from build123d import *

# Parameters (mm, degrees)
BASE_BLOCK_DEPTH        = 10
ROUND_SPIGOT_DEPTH      = 9
PROFILE_CUT_A_DEPTH     = 10
TRIANGULAR_POCKET_DEPTH = 10
PROFILE_CUT_B_SKETCH_R  = 0.5
PROFILE_CUT_B_DEPTH     = 5
SPIGOT_CHAMFER_0_5_SIZE = 0.5
SPIGOT_BORE_SKETCH_R    = 1.25
SPIGOT_BORE_DEPTH       = 12
BORE_CHAMFER_1_SIZE     = 1


with BuildPart() as part:
    # Base Block Sketch → Base Block (new body)
    with BuildSketch(Plane.XY):
        Polygon((0, 0), (10, 0), (10, -8), (0, -10), align=None)
    extrude(amount=BASE_BLOCK_DEPTH)

    # Spigot Sketch → Round Spigot (add)
    with BuildSketch(Plane.XY.offset(10)):
        with BuildLine():
            ThreePointArc((5, -0.901174016), (2, -3.901174016), (5, -6.901174016))
            Line((5, -6.901174016), (5, -3.901174016))
            Line((5, -3.901174016), (5, -0.901174016))
        make_face()
        with BuildLine():
            Line((5, -3.901174016), (5, -6.901174016))
            ThreePointArc((5, -6.901174016), (5.282604808, -6.887833442), (5.562696209, -6.847930365))
            Line((5.562696209, -6.847930365), (5, -3.901174016))
        make_face()
        with BuildLine():
            Line((5, -3.901174016), (5.562696209, -6.847930365))
            ThreePointArc((5.562696209, -6.847930365), (7.311718909, -5.813229373), (8, -3.901174016))
            ThreePointArc((8, -3.901174016), (7.121320344, -1.779853673), (5, -0.901174016))
            Line((5, -0.901174016), (5, -3.901174016))
        make_face()
    extrude(amount=ROUND_SPIGOT_DEPTH)

    # Profile Cut A Sketch → Profile Cut A (cut)
    with BuildSketch(Plane.XY.offset(10)):
        Polygon((1, -9.8), (1, -3.901174016), (0, -2.901174016), (0, -10), align=None)
    extrude(amount=-PROFILE_CUT_A_DEPTH, mode=Mode.SUBTRACT)

    # Triangular Pocket Sketch → Triangular Pocket (cut)
    with BuildSketch(Plane(origin=(0, 0, 0), x_dir=(1, 0, 0), z_dir=(0, 1, 0))):
        with BuildLine():
            Line((2.650768448, -5.144949642), (3.919921658, -1.657979857))
            ThreePointArc((3.919921658, -1.657979857), (4.286037842, -1.180847956), (4.859614278, -1))
            Line((4.859614278, -1), (6.5, -1))
            ThreePointArc((6.5, -1), (7.207106781, -1.292893219), (7.5, -2))
            Line((7.5, -2), (7.5, -7.5))
            ThreePointArc((7.5, -7.5), (7.207106781, -8.207106781), (6.5, -8.5))
            Line((6.5, -8.5), (5, -8.5))
            Line((5, -8.5), (2.85777799, -8.5))
            ThreePointArc((2.85777799, -8.5), (2.038625946, -8.073576436), (1.918085369, -7.157979857))
            Line((1.918085369, -7.157979857), (2.650768448, -5.144949642))
        make_face()
    extrude(amount=-TRIANGULAR_POCKET_DEPTH, mode=Mode.SUBTRACT)

    # Profile Cut B Sketch → Profile Cut B (cut)
    with BuildSketch(Plane.ZY):
        with Locations((3, -1.5)):
            Circle(PROFILE_CUT_B_SKETCH_R)
        with Locations((6, -1.5)):
            Circle(PROFILE_CUT_B_SKETCH_R)
    extrude(amount=-PROFILE_CUT_B_DEPTH, mode=Mode.SUBTRACT)

    # Spigot Chamfer 0.5
    spigot_chamfer_0_5_edges = [part.edges().sort_by_distance(p)[0] for p in [
        (4.437303791, -0.954417668, 10),
    ]]
    chamfer(spigot_chamfer_0_5_edges, length=SPIGOT_CHAMFER_0_5_SIZE)

    # Spigot Bore Sketch → Spigot Bore (cut)
    with BuildSketch(Plane.XY.offset(19)):
        with Locations((5, -3.901174016)):
            Circle(SPIGOT_BORE_SKETCH_R)
    extrude(amount=-SPIGOT_BORE_DEPTH, mode=Mode.SUBTRACT)

    # Bore Chamfer 1
    bore_chamfer_1_edges = [part.edges().sort_by_distance(p)[0] for p in [
        (3.75, -3.901174016, 19),
    ]]
    chamfer(bore_chamfer_1_edges, length=BORE_CHAMFER_1_SIZE)


solid = part.part
The model under review builds one solid part; all positions refer to its coordinate system, in mm. A direction names the side the tool comes from. Round coordinates to 2 decimals unless told otherwise and drop trailing zeros. Loops run counter-clockwise (first coordinate to the right, second up) from the corner with the lowest first, then second, coordinate; pieces in that order, holes last. Notation, with made-up numbers: M 1.5,39.25 L 16.5,39.25 A10 ccw 16.5,57.25 Z; hole C 31,59.5 d11. An arc over 180 degrees is marked long. Answer as CSV lines item,"result". Start each with the question number.
Item 1: Consider section A-A (z = 6). Write out the cut boundary in (x, y).
Item 2: Consider section C-C (x = 0.75). Write out the cut boundary in (y, z).
Item 3: For faces 1 (the face through (7, -7, 10)), 2 (the face through (2.7, 0, 3.8)), 3 (the face through (2, -1, 3)), 4 (the face through (6, -4, 1)), 5 (the face through (1, -7, 5)), list the 3-axis set-ups (+Z, -Z, +X, -X, +Y, -Y) from which the entire face can be reached by the end or side of a thin tool; tool diameter is ignored.
Item 4: Consider section B-B (z = 17.75). Write out the cut boundary in (x, y), then the cut area to 3 significant figures.
Item 5: Wall thickness on line 1 (Z direction, x = 1.55, y = -1.5); line 2 (Z direction, x = 6, y = -0.25); line 3 (Y direction, x = 5, z = 15.5): over which ranges is each line inside the solid? List them lowest first. Write a range as [from, to].
Item 6: Mouldability with a two-part tool opening along Y and no side actions: class faces 6 (the face through (7.215, -4.289, 8.199)), 7 (the face through (1, -1, 6)), 8 (the face through (0.5, -3.4, 5.1)), 9 (the face through (6.192, -3.526, 13.317)) as released by +Y, released by -Y, zero draft, split by the parting line, or undercut.
Item 7: Consider section D-D (x = 4.25). State how many separate pieces and enclosed holes the cut face has, then the cut area to 3 significant figures.
Item 8: Insertion check: P1, Ø1, axis at x = 6, y = -8, coming from the +Z side; P2, Ø4, axis at x = 4, z = 11, coming from the -Y side; P3, Ø1.6, axis at y = -5, z = 4, coming from the -X side. Each pin has a flat end and moves straight along its axis. Give the tip position at first contact, or say it passes through.
Answer:
1,outline,"M 0,-2.9 L 1,-3.9 L 1,-9.8 L 2.34,-9.53 L 2.34,-2 L 0,-2 Z; M 0,-1 L 2.34,-1 L 2.34,0 L 0,0 Z; M 7.5,-8.5 L 10,-8 L 10,0 L 7.5,0 Z"
2,outline,"M -3.65,0 L 0,0 L 0,10 L -3.65,10 Z; hole C -1.5,3 d1; hole C -1.5,6 d1"
3,face 1,"+Z"
3,face 2,"+Z, -Z, +X, -X, +Y"
3,face 3,"-X"
3,face 4,"+Y, -Y"
3,face 5,"+Z, -Z, -X, -Y"
4,outline,"C 5,-3.9 d6; hole C 5,-3.9 d2.5"
4,area,"23.4 mm^2"
5,line 1,"z = [0, 2.5], [3.5, 5.5], [6.5, 10]"
5,line 2,"z = [0, 1], [8.5, 10]"
5,line 3,"y = [-6.9, -5.15], [-2.65, -0.9]"
6,face 6,"zero draft"
6,face 7,"undercut"
6,face 8,"released by -Y"
6,face 9,"undercut"
7,separate pieces,"3"
7,enclosed holes,"0"
7,area,"55.2 mm^2"
8,P1,"stops at z = 10"
8,P2,"stops at y = -9.55"
8,P3,"stops at x = 1"
